from build123d import *

# Parameters (mm, degrees)
SKETCH_1_R                = 30
EXTRUDE_1_DEPTH           = 20
SKETCH_2_R                = 15
EXTRUDE_2_DEPTH           = 115
SKETCH_3_W                = 15
SKETCH_3_H                = 65.275195259
CUT_EXTRUDE_1_DEPTH       = 50
SKETCH_4_W                = 11.214536165
SKETCH_4_H                = 73.146220951
CUT_EXTRUDE_2_DEPTH       = 25
HOLE_WIZARD_10_5_10_5_1_D = 10.5
HOLE_WIZARD_M3_1_D        = 2.5


with BuildPart() as part:
    # 草图1 → 凸台-拉伸1 (new body)
    with BuildSketch(Plane(origin=(0, 0, 0), x_dir=(1, 0, 0), z_dir=(0, 1, 0))):
        with Locations(Location((0, 0, 0), (0, 0, 270))):
            Circle(SKETCH_1_R)
    extrude(amount=EXTRUDE_1_DEPTH)

    # 草图2 → 凸台-拉伸2 (add)
    with BuildSketch(Plane(origin=(0, 20, 0), x_dir=(1, 0, 0), z_dir=(0, 1, 0))):
        with Locations(Location((0, 0, 0), (0, 0, 270))):
            Circle(SKETCH_2_R)
    extrude(amount=EXTRUDE_2_DEPTH)

    # 草图3 → 切除-拉伸1 (cut, symmetric)
    with BuildSketch(Plane.XY):
        with Locations((0, 112.63759763)):
            Rectangle(SKETCH_3_W, SKETCH_3_H)
    extrude(amount=CUT_EXTRUDE_1_DEPTH, both=True, mode=Mode.SUBTRACT)

    # 草图4 → 切除-拉伸2 (cut, symmetric)
    with BuildSketch(Plane.XY):
        with Locations((19.107268082, 114.573110476)):
            Rectangle(SKETCH_4_W, SKETCH_4_H)
        with Locations((-19.107268082, 114.573110476)):
            Rectangle(SKETCH_4_W, SKETCH_4_H)
    extrude(amount=CUT_EXTRUDE_2_DEPTH, both=True, mode=Mode.SUBTRACT)

    # Ø10.5 (10.5) 直径孔1 (through all)
    with Locations(Plane(origin=(13.5, 0, 0), x_dir=(0, 0, -1), z_dir=(1, 0, 0))):
        with Locations((0, 97.25), (0, 122.25)):
            Hole(HOLE_WIZARD_10_5_10_5_1_D / 2)

    # M3 螺纹孔1 (through all)
    with Locations(Plane.ZY.offset(13.5)):
        with Locations((0, 81.4)):
            Hole(HOLE_WIZARD_M3_1_D / 2)


solid = part.part
Build history of the part. All positions in model axes, mm. A direction names the side the tool comes from. Give positions to 0.01 mm unless a question says otherwise; leave off trailing zeros. Loops run counter-clockwise (first coordinate to the right, second up) from the corner with the lowest first, then second, coordinate; pieces in that order, holes last. Notation, with made-up numbers: (-32, 28.5) - (-21, 28.5) arc R22 cw to (-21, 43.5) - close; hole circle Ø10 at (-29.75, 18). An arc over 180 degrees is marked (long way). Write item = value, one per line. Start each with the question number.
1) Band-saw the part on D-D on y = 38. Give the cut face in (x, z), plus the area to 3 significant figures.
2) Band-saw the part on C-C on z = -9. Give the cut face in (x, y), plus the area to 3 significant figures.
3) Band-saw the part on B-B on x = 0. Give the cut face in (y, z).
4) Band-saw the part on A-A on y = 97.25. Give the cut face in (x, z).
5) Drop flat-ended pins along their axis: pin 1 Ø8 at (y, z) = (102, -5) entering from +X; pin 2 Ø4 at (x, y) = (-10, 89) entering from +Z; pin 3 Ø6.5 at (y, z) = (122.25, 0) entering from +X; pin 4 Ø6 at (y, z) = (79.5, 3) entering from +X. Give the stop position or say it passes through.
6) Pull direction X, two halves, no side cores. Call faces 6 (the cylindrical face through (10.46, 126.68, 2.82)), 7 (the flat face through (-13.5, 106, 0)), 8 (the flat face through (-7.5, 107, 0)), 9 (the flat face through (7.5, 107, 0)): +X half, -X half, draft (parallel to the pull), parting line (faces both ways), or undercut.
7) Probe probe 1 along Y at (x, z) = (-11, 0); probe 2 along Y at (x, z) = (12.5, 0.5); probe 3 along Y at (x, z) = (-18, 1). List the from-to ranges inside material, lowest first. Write a range as from..to.
8) Tool access for faces 1 (the flat face through (0, 80, 0)), 2 (the flat face through (14, 20, 6)), 3 (the flat face through (13.5, 106, 0)), 4 (the cylindrical face through (1.32, 9.86, -29.97)), 5 (the flat face through (0, 0, 0)): list every direction of +Z, -Z, +X, -X, +Y, -Y with a clear straight run to the whole face (end or side of a thin tool).
Final values:
q1.outline = circle Ø30 at (0, 0)
q1.area = 707 mm²
q2.outline = (-28.62, 0) - (28.62, 0) - (28.62, 20) - (12, 20) - (12, 135) - (7.5, 135) - (7.5, 80) - (-7.5, 80) - (-7.5, 135) - (-12, 135) - (-12, 20) - (-28.62, 20) - close
q2.area = 3,080 mm²
q3.outline = (0, -30) - (20, -30) - (20, -15) - (80, -15) - (80, 15) - (20, 15) - (20, 30) - (0, 30) - close
q4.outline = (-13.5, -6.54) arc R15 ccw to (-7.5, -12.99) - (-7.5, -5.25) - (-13.5, -5.25) - close; (-13.5, 5.25) - (-7.5, 5.25) - (-7.5, 12.99) arc R15 ccw to (-13.5, 6.54) - close; (7.5, -12.99) arc R15 ccw to (13.5, -6.54) - (13.5, -5.25) - (7.5, -5.25) - close; (7.5, 5.25) - (13.5, 5.25) - (13.5, 6.54) arc R15 ccw to (7.5, 12.99) - close
q5.pin_1 = 13.5
q5.pin_2 = 12.69
q5.pin_3 = through
q5.pin_4 = 14.99
q6.face_6 = draft
q6.face_7 = -X half
q6.face_8 = undercut
q6.face_9 = undercut
q7.probe_1 = 0..80.15, 82.65..92, 102.5..117, 127.5..135
q7.probe_2 = 0..80.25, 82.55..92.02, 102.48..117.02, 127.48..135
q7.probe_3 = 0..20
q8.face_1 = +Z, -Z, +Y
q8.face_2 = +Y
q8.face_3 = +Z, -Z, +X, +Y
q8.face_4 = +Y, -Y
q8.face_5 = +Z, -Z, +X, -X, -Y
